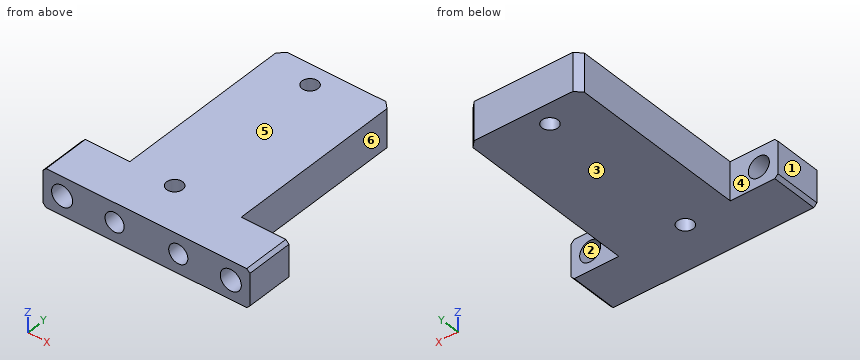
from build123d import *

# Parameters (mm, degrees)
SKETCH_1_W           = 35
SKETCH_1_H           = 73
EXTRUDE_1_DEPTH      = 6
SKETCH_2_W           = 65
SKETCH_2_H           = 12
EXTRUDE_2_DEPTH      = 15
HOLE_WIZARD_M6_1_D   = 6.6
F_6_0MM_1_D          = 6
F_6_0MM_1_DEPTH      = 15
F_6_0MM_1_TIP        = 1.802581857
HOLE_WIZARD_M6_1_2_D = 5
CHAMFER_1_SIZE       = 1
CHAMFER_2_SIZE       = 2


with BuildPart() as part:
    # 草图1 → 凸台-拉伸1 (new, symmetric)
    with BuildSketch(Plane.XY):
        Rectangle(SKETCH_1_W, SKETCH_1_H)
    extrude(amount=EXTRUDE_1_DEPTH, both=True)

    # 草图2 → 凸台-拉伸2 (add)
    with BuildSketch(Plane.XZ.offset(36.5)):
        Rectangle(SKETCH_2_W, SKETCH_2_H)
    extrude(amount=-EXTRUDE_2_DEPTH)

    # Hole Wizard M6 _1 (through all)
    with Locations(Plane(origin=(0, -21.5, 0), x_dir=(1, 0, 0), z_dir=(0, 1, 0))):
        with Locations((-26.5, 0), (26.5, 0)):
            Hole(HOLE_WIZARD_M6_1_D / 2)

    # Ø6.0mm 暗销孔1
    with Locations(Plane(origin=(0, -36.5, 0), x_dir=(-1, 0, 0), z_dir=(0, -1, 0))):
        with Locations((10, 0), (-10, 0)):
            Hole(F_6_0MM_1_D / 2, depth=F_6_0MM_1_DEPTH)
            with Locations((0, 0, -(F_6_0MM_1_DEPTH + F_6_0MM_1_TIP / 2))):  # 118° drill point
                Cone(0, F_6_0MM_1_D / 2, F_6_0MM_1_TIP, mode=Mode.SUBTRACT)

    # Hole Wizard M6 _1 2 (through all)
    with Locations(Plane(origin=(0, 0, -6), x_dir=(-1, 0, 0), z_dir=(0, 0, -1))):
        with Locations((3, -22), (3, 30)):
            Hole(HOLE_WIZARD_M6_1_2_D / 2)

    # 倒角1
    chamfer_1_edges = [part.edges().sort_by_distance(p)[0] for p in [
        (-32.5, -29, 6),
        (32.5, -29, -6),
        (-32.5, -29, -6),
        (32.5, -29, 6),
    ]]
    chamfer(chamfer_1_edges, length=CHAMFER_1_SIZE)

    # 倒角2
    chamfer_2_edges = [part.edges().sort_by_distance(p)[0] for p in [
        (-17.5, 36.5, 0),
        (17.5, 36.5, 0),
    ]]
    chamfer(chamfer_2_edges, length=CHAMFER_2_SIZE)


solid = part.part
Check sheet for the modelled part. Datum: model origin and axes. Units: mm. Face numbers are marked on the shaded views. A direction names the side the tool comes from. Coordinates: 2 decimals unless noted, no trailing zeros. Write each loop counter-clockwise with the first axis right and the second up, starting at its lowest first coordinate (ties: lowest second). Pieces come first, ordered by that corner, then holes.
Item 1: Access from +Z, -Z, +X, -X, +Y, -Y to the whole of each face (thin tool, end or side, straight path). Record for the marked faces 4, 5 and 6.
Numbers:
face 4: +Z, -Z, -X, +Y
face 5: +Z, +X, -X, +Y, -Y
face 6: +Z, -Z, +X, +Y
Item 2: Scan lines: probe 1 along Z at (x, y) = (-10, -28); probe 2 along X at (y, z) = (18.5, 4); probe 3 along Y at (x, z) = (21.5, 0.75). Record each from-to range of solid material in increasing order.
Numbers:
probe 1: z = -6 to -3, 3 to 6
probe 2: x = -17.5 to 17.5
probe 3: y = -36.5 to -21.5
Item 3: Cross-section at B-B on x = 25.5. Record the boundary of the cut face in (y, z), then the cut area to 3 significant figures.
Numbers:
outline: (-36.5, -6) - (-21.5, -6) - (-21.5, -3.14) - (-36.5, -3.14) - close; (-36.5, 3.14) - (-21.5, 3.14) - (-21.5, 6) - (-36.5, 6) - close
area: 85.7 mm2
Item 4: Depth check by flat-ended pin: pin 1 Ø3 at (y, z) = (-4, -4.5) entering from -X; pin 2 Ø6 at (y, z) = (8, -1.5) entering from +X; pin 3 Ø3 at (x, z) = (23, 1.5) entering from +Y. Enter the tip coordinate at first touch or a pass-through.
Numbers:
pin 1: stops at x = -17.5
pin 2: stops at x = 17.5
pin 3: stops at y = -21.5
Item 5: Cross-section at C-C on y = 14. Record the boundary of the cut face in (x, z), then the cut area to 3 significant figures.
Numbers:
outline: (-17.5, -6) - (17.5, -6) - (17.5, 6) - (-17.5, 6) - close
area: 420 mm2
Item 6: Mould release check, pull along X, two halves, no side actions. Record for the marked faces 1, 2 and 3: released by +X, released by -X, zero draft, split by the parting line, or undercut.
Numbers:
face 1: released by -X
face 2: undercut
face 3: zero draft
Item 7: Cross-section at A-A on x = -26.5. Record the boundary of the cut face in (y, z), then the cut area to 3 significant figures.
Numbers:
outline: (-36.5, -6) - (-21.5, -6) - (-21.5, -3.3) - (-36.5, -3.3) - close; (-36.5, 3.3) - (-21.5, 3.3) - (-21.5, 6) - (-36.5, 6) - close
area: 81.0 mm2
